```python
from build123d import *

# Parameters (mm, degrees)
SKETCH1_R           = 3
BOSS_EXTRUDE1_DEPTH = 30
SKETCH2_W           = 24
SKETCH2_H           = 30
SKETCH2_W_2         = 18
SKETCH2_H_2         = 40
CUT_EXTRUDE1_DEPTH  = 42
CUT_EXTRUDE2_DEPTH  = 3
CUT_EXTRUDE3_START  = -30
CUT_EXTRUDE3_DEPTH  = 3
FILLET1_R           = 1
CUT_EXTRUDE4_DEPTH  = 10


with BuildPart() as part:
    # Sketch1 → Boss-Extrude1 (new body)
    with BuildSketch(Plane.XY):
        with BuildLine():
            Line((-7.5, 65), (-7.5, 0))
            ThreePointArc((-7.5, 0), (-4.820907073, -5.745333323), (1.302361333, -7.386058148))
            Line((1.302361333, -7.386058148), (7.5, -6.293247234))
            Line((7.5, -6.293247234), (7.5, 65))
            ThreePointArc((7.5, 65), (0, 72.5), (-7.5, 65))
        make_face()
        Circle(SKETCH1_R, mode=Mode.SUBTRACT)
        with Locations((0, 65)):
            Circle(SKETCH1_R, mode=Mode.SUBTRACT)
    extrude(amount=BOSS_EXTRUDE1_DEPTH)

    # Sketch2 → Cut-Extrude1 (cut)
    with BuildSketch(Plane(origin=(7.5, 0, 0), x_dir=(0, 0, -1), z_dir=(1, 0, 0))):
        with Locations((-15, -7.386058148)):
            Rectangle(SKETCH2_W, SKETCH2_H)
        with Locations((-15, 72.5)):
            Rectangle(SKETCH2_W_2, SKETCH2_H_2)
    extrude(amount=-CUT_EXTRUDE1_DEPTH, mode=Mode.SUBTRACT)

    # Sketch3<2> → Cut-Extrude2 (cut)
    with BuildSketch(Plane.XY.offset(30)):
        Polygon((-7.5, 45), (0, 49.686520139), (7.5, 45), (7.5, 48.622120254), (18.624271708, 48.622120254), (18.624271708, 113.745401459), (-18.624271708, 113.745401459), (-18.624271708, 48.622120254), (-7.5, 48.622120254), align=None)
    extrude(amount=-CUT_EXTRUDE2_DEPTH, mode=Mode.SUBTRACT)

    # 草图3<2> → Cut-Extrude3 (cut)
    with BuildSketch(Plane.XY.offset(30).offset(CUT_EXTRUDE3_START)):
        Polygon((-7.5, 45), (0, 49.686520139), (7.5, 45), (7.5, 48.622120254), (18.624271708, 48.622120254), (18.624271708, 113.745401459), (-18.624271708, 113.745401459), (-18.624271708, 48.622120254), (-7.5, 48.622120254), align=None)
    extrude(amount=CUT_EXTRUDE3_DEPTH, mode=Mode.SUBTRACT)

    # Fillet1
    fillet1_edges = [part.edges().sort_by_distance(p)[0] for p in [
        (0, 49.686520139, 1.5),
        (0, 49.686520139, 28.5),
    ]]
    fillet(fillet1_edges, radius=FILLET1_R)

    # Sketch4 → Cut-Extrude4 (cut)
    with BuildSketch(Plane(origin=(7.5, 0, 0), x_dir=(0, 0, -1), z_dir=(1, 0, 0))):
        Polygon((-3, -16.386058148), (-27, -16.386058148), (-27, 31.613941852), (-24, 31.613941852), (-24, 73.386058148), (-6, 73.386058148), (-6, 31.613941852), (-3, 31.613941852), align=None)
    extrude(amount=-CUT_EXTRUDE4_DEPTH, mode=Mode.SUBTRACT)


solid = part.part
```
Read the model definition and answer for the solid it produces. Units are mm, in the model's axes. A direction names the side the tool comes from. Coordinates: 2 decimals unless noted, no trailing zeros. Loops run counter-clockwise (first coordinate to the right, second up) from the corner with the lowest first, then second, coordinate; pieces in that order, holes last.
(1) Flat-ended cylindrical pins translate along their axes: pin 1 Ø8 at (x, y) = (0, 0) entering from -Z; pin 2 Ø3.5 at (x, z) = (4, 4) entering from -Y; pin 3 Ø4.5 at (x, y) = (0, 58) entering from -Z; pin 4 Ø0.9 at (x, z) = (2.5, 26) entering from -Y. Find the tip coordinate at first contact, or state that the pin passes through.
Solution:
pin 1: stops at z = 0
pin 2: stops at y = -7.16
pin 3: stops at z = 3
pin 4: stops at y = 31.61
(2) The part is cut by section D-D (x = 4.5). Determine the outline of the cut face in (y, z).
Solution:
outline: (-6.82, 0) - (46.87, 0) - (46.87, 3) - (71, 3) - (71, 6) - (31.61, 6) - (31.61, 3) - (-6.82, 3) - close; (-6.82, 27) - (31.61, 27) - (31.61, 24) - (71, 24) - (71, 27) - (46.87, 27) - (46.87, 30) - (-6.82, 30) - close
(3) The mould has two halves that part along Y. Classify faces 6 (the face through (-4.891, -5.686, 1.479)), 7 (the face through (-3, 0, 28)), 8 (the face through (-4.06, 47.15, 28.52)): released by +Y, released by -Y, zero draft, split by the parting line, or undercut.
Solution:
face 6: released by -Y
face 7: undercut
face 8: released by +Y
(4) The part is cut by section C-C (y = 17). Determine the outline of the cut face in (x, z), and give its area (3 significant figures).
Solution:
outline: (-7.5, 0) - (7.5, 0) - (7.5, 3) - (-2.5, 3) - (-2.5, 27) - (7.5, 27) - (7.5, 30) - (-7.5, 30) - close
area: 210 mm2
(5) The part is cut by section A-A (y = 58). Determine the outline of the cut face in (x, z), and give its area (3 significant figures).
Solution:
outline: (-7.5, 3) - (7.5, 3) - (7.5, 6) - (-7.5, 6) - close; (-7.5, 24) - (7.5, 24) - (7.5, 27) - (-7.5, 27) - close
area: 90.0 mm2
(6) Consider line 1 along X through (y, z) = (65, 25.65); line 2 along Z through (x, y) = (6, 12.5); line 3 along Z through (x, y) = (5.75, 35). Determine where each line is inside the solid, lowest interval first.
Solution:
line 1: x = -7.5 to -3, 3 to 7.5
line 2: z = 0 to 3, 27 to 30
line 3: z = 0 to 6, 24 to 30
(7) A tool of negligible diameter and unlimited length cuts with its end or side. For faces 1 (the face through (-4.06, 47.15, 1.48)), 2 (the face through (3.966, 47.208, 28.521)), 3 (the face through (2, 12, 3)), 4 (the face through (2, 52, 6)), 5 (the face through (3.966, 47.208, 1.479)), from which of +Z, -Z, +X, -X, +Y, -Y can it reach the whole face along a straight path? Write none if from no direction.
Solution:
face 1: -Z, -X, +Y
face 2: +Z, +X, +Y
face 3: +X, -Y
face 4: +X, +Y
face 5: -Z, +X, +Y
(8) The part is cut by section B-B (z = 28.25). Determine the outline of the cut face in (x, y), and give its area (3 significant figures).
Solution:
outline: (-7.5, 0) arc R7.5 ccw to (1.3, -7.39) - (7.5, -6.29) - (7.5, 45) - (0.53, 49.36) arc R1 ccw to (-0.53, 49.36) - (-7.5, 45) - close; hole circle Ø6 at (0, 0)
area: 778 mm2
